```python
from build123d import *


with BuildPart() as part:
    # Sketch1 → Revolve1 (revolve)
    with BuildSketch(Plane(origin=(0, 0, 0), x_dir=(1, 0, 0), z_dir=(0, 1, 0)), mode=Mode.PRIVATE) as revolve1_sk:
        Polygon((0, 150), (0, 163), (14, 163), (14, 177), (0, 177), (0, 189), (14, 189), (14, 203), (0, 203), (0, 219.5), (45, 219.5), (45, 227.5), (59, 227.5), (59, 219.5), (71, 219.5), (71, 200), (30, 200), (30, 150), align=None)
    revolve(revolve1_sk.sketch.rotate(Axis((0, 0, 0), (1, 0, 0)), 180), axis=Axis((0, 0, 0), (1, 0, 0)))


solid = part.part
```
Geometry check sheet. Reference: the model listing, model coordinates, mm. A direction names the side the tool comes from. Give positions to 0.01 mm unless a question says otherwise; leave off trailing zeros. Loops run counter-clockwise (first coordinate to the right, second up) from the corner with the lowest first, then second, coordinate; pieces in that order, holes last. Notation, with made-up numbers: M 37,72.25 L 62,72.25 A32 cw 62,107.25 Z; hole C -23.5,-26 d5. An arc over 180 degrees is marked long. Answer as CSV lines item,"result".
Item 1: Access from +Z, -Z, +X, -X, +Y, -Y to the whole of each face (thin tool, end or side, straight path). Record for faces 4 (the flat face through (0, 132, -72)), 5 (the flat face through (14, 143.4, -77.84)), 6 (the flat face through (59, -186, -119)).
Values:
face 4,"+Z, -Z, -X, +Y, -Y"
face 5,"-X"
face 6,"+X"
Item 2: Release check for a two-part mould opening along Z. For faces 1 (the cylindrical face through (65.08, 214.28, -47.58)), 2 (the flat face through (45, -186, 119)), 3 (the cylindrical face through (7.1, 62.43, 150.57)) record: pulls with the +Z half, pulls with the -Z half, needs draft (parallel to the pull), parting line crosses it, or undercut.
Values:
face 1,"parting line crosses it"
face 2,"needs draft"
face 3,"undercut"
Item 3: Cross-section at A-A on x = 37.5. Record the cut outline in (y, z), and give its area (3 significant figures).
Values:
outline,"C 0,0 d439; hole C 0,0 d400"
area,"25,700 mm²"
Item 4: Depth check by flat-ended pin: P1, Ø1, axis at x = 25.5, y = 178.5, coming from the -Z side; P2, Ø1, axis at x = 16.5, z = -15.5, coming from the +Y side; P3, Ø4, axis at x = 17.5, z = 170, coming from the -Y side. Enter the tip coordinate at first touch or a pass-through.
Values:
P1,"stops at z = -128.44"
P2,"stops at y = 218.99"
P3,"stops at y = -141.27"
Item 5: Material ranges on line 1 (Y direction, x = 13, z = 0); line 2 (Y direction, x = 16.5, z = 0); line 3 (Y direction, x = 58.5, z = 0), recorded low to high.
Values:
line 1,"y = -219.5 to -203, -189 to -177, -163 to -150, 150 to 163, 177 to 189, 203 to 219.5"
line 2,"y = -219.5 to -150, 150 to 219.5"
line 3,"y = -227.5 to -200, 200 to 227.5"
